Can you work these out from the model? Positions are in its coordinate system, mm. Round coordinates to 2 decimals unless told otherwise and drop trailing zeros. Loops run counter-clockwise (first coordinate to the right, second up) from the corner with the lowest first, then second, coordinate; pieces in that order, holes last. Notation, with made-up numbers: M 77.5,57.25 L 131.5,57.25 A18 ccw 131.5,91.25 Z; hole C -17.5,40.25 d3. An arc over 180 degrees is marked long. Return JSON: item names as keys, results as strings.
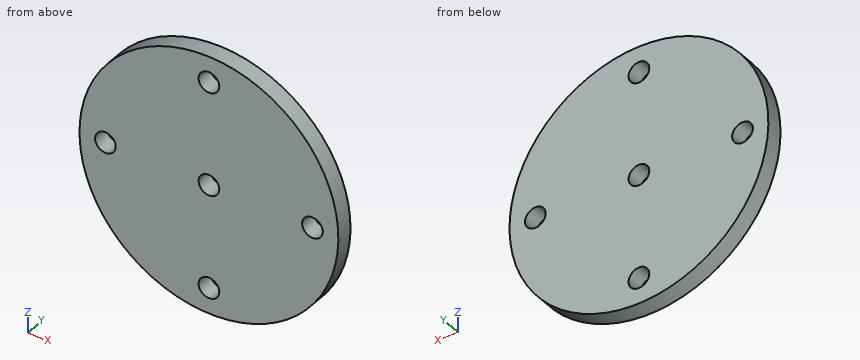
```python
from build123d import *

# Parameters (mm, degrees)
SKETCH1_R           = 75
BOSS_EXTRUDE1_DEPTH = 10
SKETCH2_R           = 6
CUT_EXTRUDE1_DEPTH  = 107.536378763


with BuildPart() as part:
    # Sketch1 → Boss-Extrude1 (new body)
    with BuildSketch(Plane(origin=(0, 0, 0), x_dir=(1, 0, 0), z_dir=(0, 1, 0))):
        with Locations(Location((0, 0, 0), (0, 0, 270))):
            Circle(SKETCH1_R)
    extrude(amount=BOSS_EXTRUDE1_DEPTH)

    # Sketch2 → Cut-Extrude1 (cut, through all)
    with BuildSketch(Plane(origin=(0, 10, 0), x_dir=(1, 0, 0), z_dir=(0, 1, 0))):
        with Locations(Location((0, 60, 0), (0, 0, 270))):
            Circle(SKETCH2_R)
        with Locations(Location((0, 0, 0), (0, 0, 270))):
            Circle(SKETCH2_R)
        with Locations(Location((0, -60, 0), (0, 0, 270))):
            Circle(SKETCH2_R)
        with Locations(Location((-60, 0, 0), (0, 0, 270))):
            Circle(SKETCH2_R)
        with Locations(Location((60, 0, 0), (0, 0, 270))):
            Circle(SKETCH2_R)
    extrude(amount=-CUT_EXTRUDE1_DEPTH, mode=Mode.SUBTRACT)


solid = part.part
```
Q1. I'm going to push flat-ended pins straight in: pin 1 Ø1 at (x, y) = (-5.5, 8) entering from -Z; pin 2 Ø6 at (x, y) = (41, 2) entering from +Z; pin 3 Ø5 at (y, z) = (2.5, 46.5) entering from -X. Where does each tip first touch, or does it pass through?
Results:
{"pin 1": "stops at z = -74.83", "pin 2": "stops at z = 64.66", "pin 3": "stops at x = -60.74"}
Q2. Suppose I cut it at B-B, the plane x = -60. Please give me the cut outline in (y, z).
Results:
{"outline": "M 0,-45 L 10,-45 L 10,-6 L 0,-6 Z; M 0,6 L 10,6 L 10,45 L 0,45 Z"}
Q3. If I drill on line 1 along X through (y, z) = (3.5, 0); line 2 along Z through (x, y) = (5.5, 0.75); line 3 along Z through (x, y) = (-3, 3.25), over which ranges is the centre line in solid material (lowest first)?
Results:
{"line 1": "x = -75 to -66, -54 to -6, 6 to 54, 66 to 75", "line 2": "z = -74.8 to -62.4, -57.6 to -2.4, 2.4 to 57.6, 62.4 to 74.8", "line 3": "z = -74.94 to -65.2, -54.8 to -5.2, 5.2 to 54.8, 65.2 to 74.94"}
Q4. Suppose I cut it at D-D, the plane z = 60. Please give me the cut outline in (x, y), plus the area to 3 significant figures.
Results:
{"outline": "M -45,0 L -6,0 L -6,10 L -45,10 Z; M 6,0 L 45,0 L 45,10 L 6,10 Z", "area": "780 mm2"}
Q5. Suppose I cut it at C-C, the plane x = 0. Please give me the cut outline in (y, z).
Results:
{"outline": "M 0,-75 L 10,-75 L 10,-66 L 0,-66 Z; M 0,-54 L 10,-54 L 10,-6 L 0,-6 Z; M 0,6 L 10,6 L 10,54 L 0,54 Z; M 0,66 L 10,66 L 10,75 L 0,75 Z"}
Q6. Suppose I cut it at A-A, the plane z = 0. Please give me the cut outline in (x, y).
Results:
{"outline": "M -75,0 L -66,0 L -66,10 L -75,10 Z; M -54,0 L -6,0 L -6,10 L -54,10 Z; M 6,0 L 54,0 L 54,10 L 6,10 Z; M 66,0 L 75,0 L 75,10 L 66,10 Z"}
